For this review, take the finished solid that the model builds, in its own axes (mm). Face numbers are marked on the shaded views. A direction names the side the tool comes from. Coordinates: 2 decimals unless noted, no trailing zeros. Write each loop counter-clockwise with the first axis right and the second up, starting at its lowest first coordinate (ties: lowest second). Pieces come first, ordered by that corner, then holes.
1) To check wall thickness, follow line 1 along Z through (x, y) = (0, 6); line 2 along Z through (x, y) = (0, 24); line 3 along X through (y, z) = (38, 6). State the ranges of each line that lie inside material, in increasing order.
2) Insertion check: P1, Ø8, axis at y = 28.5, z = 8, coming from the -X side; P2, Ø6, axis at x = -5.5, y = 36.5, coming from the +Z side; P3, Ø13, axis at x = 4.5, z = -4, coming from the -Y side. Each pin has a flat end and moves straight along its axis. Give the tip position at first contact, or say it passes through.
3) We need section A-A on z = 0. Write out the cut boundary in (x, y).
4) Mouldability with a two-part tool opening along Z and no side actions: class the marked faces 1, 2 and 3 as pulls with the +Z half, pulls with the -Z half, needs draft (parallel to the pull), parting line crosses it, or undercut.
5) We need section B-B on y = 18. Write out the cut boundary in (x, z).
6) We need section D-D on y = 6. Write out the cut boundary in (x, z), then the cut area to 3 significant figures.
7) We need section C-C on x = 0. Write out the cut boundary in (y, z), then the cut area to 3 significant figures.
8) For the marked faces 4 and 5, list the 3-axis set-ups (+Z, -Z, +X, -X, +Y, -Y) from which the entire face can be reached by the end or side of a thin tool; tool diameter is ignored.
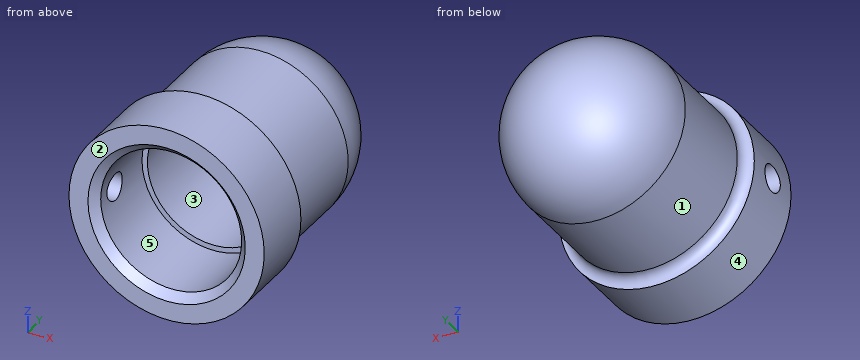
from build123d import *

# Parameters (mm, degrees)
SKETCH3_R          = 2.5
CUT_EXTRUDE1_DEPTH = 40
CHAMFER1_SIZE      = 1.5


with BuildPart() as part:
    # Sketch2 → Revolve1 (revolve)
    with BuildSketch(Plane.XY, mode=Mode.PRIVATE) as revolve1_sk:
        with BuildLine():
            Line((-16, 31), (-16, 14))
            ThreePointArc((-16, 14), (-16.585786438, 12.585786438), (-18, 12))
            Line((-18, 12), (-18, 0))
            Line((-18, 0), (-13, 0))
            Line((-13, 0), (-13, 15))
            Line((-13, 15), (-12, 15))
            Line((-12, 15), (-12, 31))
            ThreePointArc((-12, 31), (-8.485281374, 39.485281374), (0, 43))
            Line((0, 43), (0, 47))
            ThreePointArc((0, 47), (-11.313708499, 42.313708499), (-16, 31))
        make_face()
    revolve(revolve1_sk.sketch.rotate(Axis((0, -51.943033939, 0), (0, 1, 0)), 180), axis=Axis((0, -51.943033939, 0), (0, 1, 0)))

    # Sketch3 → Cut-Extrude1 (cut)
    with BuildSketch(Plane(origin=(0, 0, 0), x_dir=(0, 0, -1), z_dir=(1, 0, 0))):
        with Locations((0, 6)):
            Circle(SKETCH3_R)
    extrude(amount=-CUT_EXTRUDE1_DEPTH, mode=Mode.SUBTRACT)

    # Chamfer1
    chamfer1_edges = [part.edges().sort_by_distance(p)[0] for p in [
        (-13, 0, 0),
    ]]
    chamfer(chamfer1_edges, length=CHAMFER1_SIZE)


solid = part.part
Result:
1. line 1: z = -18 to -13, 13 to 18
1. line 2: z = -16 to -12, 12 to 16
1. line 3: x = -13.08 to -7.68, 7.68 to 13.08
2. P1: stops at x = -15.49
2. P2: stops at z = 15.27
2. P3: stops at y = 15
3. outline: (-18, 0) - (-14.5, 0) - (-13, 1.5) - (-13, 3.5) - (-18, 3.5) - close; (-18, 8.5) - (-13, 8.5) - (-13, 15) - (-12, 15) - (-12, 31) arc R12 cw to (12, 31) - (12, 15) - (13, 15) - (13, 1.5) - (14.5, 0) - (18, 0) - (18, 12) arc R2 cw to (16, 14) - (16, 31) arc R16 ccw to (-16, 31) - (-16, 14) arc R2 cw to (-18, 12) - close
4. face 1: parting line crosses it
4. face 2: needs draft
4. face 3: undercut
5. outline: circle Ø32 at (0, 0); hole circle Ø24 at (0, 0)
6. outline: (-17.83, -2.5) arc R18 ccw (long way) to (-17.83, 2.5) - (-12.76, 2.5) arc R13 cw (long way) to (-12.76, -2.5) - close
6. area: 462 mm2
7. outline: (0, -18) - (12, -18) arc R2 cw to (14, -16) - (31, -16) arc R16 ccw to (31, 16) - (14, 16) arc R2 cw to (12, 18) - (0, 18) - (0, 14.5) - (1.5, 13) - (15, 13) - (15, 12) - (31, 12) arc R12 cw to (31, -12) - (15, -12) - (15, -13) - (1.5, -13) - (0, -14.5) - close
7. area: 441 mm2
8. face 4: +Y, -Y
8. face 5: -Y
